from build123d import *

# Parameters (mm, degrees)
BOSS_EXTRUDE1_DEPTH = 7.5
M16_TAPPED_HOLE1_D  = 14


with BuildPart() as part:
    # Sketch1 → Boss-Extrude1 (new, symmetric)
    with BuildSketch(Plane.XY):
        Polygon((-50, 0), (50, 0), (50, 40), (25, 85), (-25, 85), (-50, 40), align=None)
    extrude(amount=BOSS_EXTRUDE1_DEPTH, both=True)

    # M16 Tapped Hole1 (through all)
    with Locations(Plane(origin=(0, 67, 7.5), x_dir=(1, 0, 0), z_dir=(0, 0, 1))):
        with Locations((0, 0)):
            Hole(M16_TAPPED_HOLE1_D / 2)


solid = part.part
Build history of the part. All positions in model axes, mm. Coordinates: 2 decimals unless noted, no trailing zeros. Order: outer loops, then holes, each group sorted by start corner. A loop starts at its lowest first (then second) coordinate and runs counter-clockwise, first axis right, second up. Notation, with made-up numbers: M 48,72.5 L 96,72.5 A22 ccw 96,100.5 Z; hole C -37,58 d7. An arc over 180 degrees is marked long. One line per question, with ' | ' between items. Start each with the question number.
Q1. Saw through at D-D (x = 34). List the corners of the cut face in (y, z).
Q2. Two-plate mould, pull along Y, no slides. Class faces 1 (the face through (0, 85, 0)), 2 (the face through (-1, 34, -7.5)), 3 (the face through (0.91, 73.94, -0.1)): +Y half, -Y half, draft (parallel to the pull), parting line (faces both ways), or undercut.
Q3. Probe L1, parallel to Y at x = 0, z = -3; L2, parallel to Y at x = 4.5, z = -3.25; L3, parallel to X at y = 40.5, z = -2.5. List the from-to ranges inside material, lowest first. Write a range as from..to.
Q4. Saw through at A-A (x = 0). List the corners of the cut face in (y, z).
Q5. Saw through at B-B (z = -2.25). List the corners of the cut face in (x, y), then the cut area to 3 significant figures.
Q6. Saw through at C-C (y = 71). List the corners of the cut face in (x, z), then the cut area to 3 significant figures.
Q7. Flat gauge pins, fed straight in: pin 1 Ø6 at (y, z) = (50.5, 0.5) entering from -X; pin 2 Ø1 at (y, z) = (52, -1.5) entering from -X; pin 3 Ø1.5 at (y, z) = (41, -4.5) entering from -X. Where does each tip first touch, or does it go through?
Check values:
1) outline: M 0,-7.5 L 68.8,-7.5 L 68.8,7.5 L 0,7.5 Z
2) face 1: +Y half | face 2: draft | face 3: undercut
3) L1: y = 0..60, 74..85 | L2: y = 0..61.64, 72.36..85 | L3: x = -49.72..49.72
4) outline: M 0,-7.5 L 60,-7.5 L 60,7.5 L 0,7.5 Z; M 74,-7.5 L 85,-7.5 L 85,7.5 L 74,7.5 Z
5) outline: M -50,0 L 50,0 L 50,40 L 25,85 L -25,85 L -50,40 Z; hole C 0,67 d14 | area: 7,220 mm2
6) outline: M -32.78,-7.5 L -5.74,-7.5 L -5.74,7.5 L -32.78,7.5 Z; M 5.74,-7.5 L 32.78,-7.5 L 32.78,7.5 L 5.74,7.5 Z | area: 811 mm2
7) pin 1: stops at x = -45.83 | pin 2: stops at x = -43.61 | pin 3: stops at x = -49.86
